from build123d import *

# Parameters (mm, degrees)
BAR_OUTLINE_AND_HOLE_4_76_SKETCH_W = 76.2
BAR_OUTLINE_AND_HOLE_4_76_SKETCH_H = 19.05
BAR_OUTLINE_AND_HOLE_4_76_SKETCH_R = 2.38
LINK_BAR_6_35_THICK_DEPTH          = 6.35
D_HOLE_12_7_CUT_DEPTH              = 6.35


with BuildPart() as part:
    # Bar Outline and Hole Ø4.76 Sketch → Link Bar 6.35 Thick (new body)
    with BuildSketch(Plane(origin=(0, 0, 0), x_dir=(1, 0, 0), z_dir=(0, 1, 0))):
        Rectangle(BAR_OUTLINE_AND_HOLE_4_76_SKETCH_W, BAR_OUTLINE_AND_HOLE_4_76_SKETCH_H)
        with Locations(Location((-28.75, 0, 0), (0, 0, 270))):
            Circle(BAR_OUTLINE_AND_HOLE_4_76_SKETCH_R, mode=Mode.SUBTRACT)
    extrude(amount=LINK_BAR_6_35_THICK_DEPTH)

    # D-Hole Ø12.7 Sketch → D-Hole Ø12.7 Cut (cut)
    with BuildSketch(Plane(origin=(0, 6.35, 0), x_dir=(1, 0, 0), z_dir=(0, 1, 0))):
        with BuildLine():
            Line((33.34, -3.989849621), (33.34, 3.989849621))
            ThreePointArc((33.34, 3.989849621), (22.05, 0), (33.34, -3.989849621))
        make_face()
    extrude(amount=-D_HOLE_12_7_CUT_DEPTH, mode=Mode.SUBTRACT)


solid = part.part
Input: part model. Units: mm. Frame: model coordinates. Round coordinates to 2 decimals unless told otherwise and drop trailing zeros. Order: outer loops, then holes, each group sorted by start corner. A loop starts at its lowest first (then second) coordinate and runs counter-clockwise, first axis right, second up.
1. Mould query, pull axis X, two halves, no side actions, for faces 1 (the face through (38.1, 3, 0)), 2 (the face through (33.34, 3, 0)), 3 (the face through (-1, 6.35, 0)). Classes: released by +X, released by -X, zero draft, split by the parting line, or undercut.
The answers:
face 1: released by +X
face 2: undercut
face 3: zero draft
2. Pin query (flat end, axial travel): P1, Ø4, axis at x = -28.75, z = 0, coming from the -Y side. Return the tip coordinate at first contact, or that it passes through.
The answers:
P1: passes through
3. Cut plane A-A, the plane z = 0. Output: boundary loops of the cut face in (x, y), then the cut area to 3 significant figures.
The answers:
outline: (-38.1, 0) - (-31.13, 0) - (-31.13, 6.35) - (-38.1, 6.35) - close; (-26.37, 0) - (22.05, 0) - (22.05, 6.35) - (-26.37, 6.35) - close; (33.34, 0) - (38.1, 0) - (38.1, 6.35) - (33.34, 6.35) - close
area: 382 mm2
4. Cut plane B-B, the plane x = 28.4. Output: boundary loops of the cut face in (y, z) (3 decimals), then the cut area to 3 significant figures.
The answers:
outline: (0, -9.525) - (6.35, -9.525) - (6.35, -6.35) - (0, -6.35) - close; (0, 6.35) - (6.35, 6.35) - (6.35, 9.525) - (0, 9.525) - close
area: 40.3 mm2
5. Cut plane D-D, the plane x = -28.75. Output: boundary loops of the cut face in (y, z) (3 decimals).
The answers:
outline: (0, -9.525) - (6.35, -9.525) - (6.35, -2.38) - (0, -2.38) - close; (0, 2.38) - (6.35, 2.38) - (6.35, 9.525) - (0, 9.525) - close
6. Cut plane C-C, the plane y = 5. Output: boundary loops of the cut face in (x, z) (3 decimals), then the cut area to 3 significant figures.
The answers:
outline: (-38.1, -9.525) - (38.1, -9.525) - (38.1, 9.525) - (-38.1, 9.525) - close; hole circle Ø4.76 at (-28.75, 0); hole (33.34, -3.99) - (33.34, 3.99) arc R6.35 ccw (long way) to start
area: 1,310 mm2
7. Material intervals for line 1 (X direction, y = 2, z = 0); line 2 (Z direction, x = 28.4, y = 3) (3 decimals); line 3 (X direction, y = 5.25, z = -1.25), sorted ascending.
The answers:
line 1: x = -38.1 to -31.13, -26.37 to 22.05, 33.34 to 38.1
line 2: z = -9.525 to -6.35, 6.35 to 9.525
line 3: x = -38.1 to -30.78, -26.72 to 22.17, 33.34 to 38.1
